The listing builds one solid part. Answer for the finished solid, in the listing's coordinates (mm). Face numbers are marked on the shaded views. Round coordinates to 2 decimals unless told otherwise and drop trailing zeros. Loops run counter-clockwise (first coordinate to the right, second up) from the corner with the lowest first, then second, coordinate; pieces in that order, holes last. Notation, with made-up numbers: (-10.75, 46.25) -> (11.25, 46.25) arc R12 ccw to (11.25, 66.25) -> close; hole circle Ø9 at (14, 89). An arc over 180 degrees is marked (long way). Write each question's results on one line, items separated by ' | '. Start each with the question number.
(1) A flat-ended cylindrical pin translates along its axis: pin 1 (0.6 mm diameter, centred on x = 2, y = -2.5, fed in from -Z). Find the tip coordinate at first contact, or state that the pin passes through.
(2) The part is cut by section C-C (y = 0). Determine the outline of the cut face in (x, z).
(3) The part is cut by section D-D (z = 10). Determine the outline of the cut face in (x, y), plus the area to 3 significant figures.
(4) The part is cut by section A-A (x = -7). Determine the outline of the cut face in (y, z), plus the area to 3 significant figures.
(5) Straight lines are drawn through the part: probe 1 along X at (y, z) = (-2.5, 10); probe 2 along X at (y, z) = (-1.5, -1.5); probe 3 along Z at (x, y) = (7.7, 0). For each, find the intervals that lie inside material, in ascending order.
(6) Determine the mould class of the marked faces 1, 2 and 3 for opening direction Y: released by +Y, released by -Y, zero draft, split by the parting line, or undercut.
(7) The part is cut by section B-B (z = 3.5). Determine the outline of the cut face in (x, y), plus the area to 3 significant figures.
```python
from build123d import *

# Parameters (mm, degrees)
SKETCH_1_R          = 2
EXTRUDE_1_DEPTH     = 12.5
SKETCH_2_R          = 1.7
CUT_EXTRUDE_1_DEPTH = 21.863604674
CUT_EXTRUDE_2_DEPTH = 6.5


with BuildPart() as part:
    # 草图1 → 凸台-拉伸1 (new, symmetric)
    with BuildSketch(Plane(origin=(0, 0, 0), x_dir=(0, 0, -1), z_dir=(1, 0, 0))):
        with BuildLine():
            Line((0, -3), (-16, -3))
            Line((-16, -3), (-16, -1.8))
            Line((-16, -1.8), (-2.4, -1.8))
            ThreePointArc((-2.4, -1.8), (1.341640786, 2.683281573), (0, -3))
        make_face()
        Circle(SKETCH_1_R, mode=Mode.SUBTRACT)
    extrude(amount=EXTRUDE_1_DEPTH, both=True)

    # 草图2 → 切除-拉伸1 (cut, through all)
    with BuildSketch(Plane(origin=(0, -1.8, 0), x_dir=(1, 0, 0), z_dir=(0, 1, 0))):
        with Locations(Location((-7, -10, 0), (0, 0, 270))):
            Circle(SKETCH_2_R)
        with Locations(Location((7, -10, 0), (0, 0, 270))):
            Circle(SKETCH_2_R)
    extrude(amount=-CUT_EXTRUDE_1_DEPTH, mode=Mode.SUBTRACT)

    # 草图3 → 切除-拉伸2 (cut, symmetric)
    with BuildSketch(Plane(origin=(0, 0, 0), x_dir=(0, 0, -1), z_dir=(1, 0, 0))):
        with BuildLine():
            Line((-4, -3), (0, -3))
            ThreePointArc((0, -3), (1.341640786, 2.683281573), (-2.4, -1.8))
            Line((-2.4, -1.8), (-4, -1.8))
            Line((-4, -1.8), (-4, -3))
        make_face()
    extrude(amount=CUT_EXTRUDE_2_DEPTH, both=True, mode=Mode.SUBTRACT)


solid = part.part
```
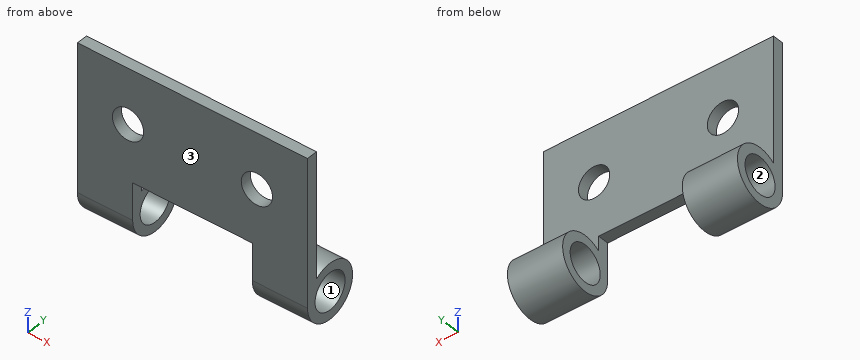
Checked values:
1) pin 1: stops at z = 4
2) outline: (-12.5, -3) -> (-6.5, -3) -> (-6.5, -2) -> (-12.5, -2) -> close; (-12.5, 2) -> (-6.5, 2) -> (-6.5, 3) -> (-12.5, 3) -> close; (6.5, -3) -> (12.5, -3) -> (12.5, -2) -> (6.5, -2) -> close; (6.5, 2) -> (12.5, 2) -> (12.5, 3) -> (6.5, 3) -> close
3) outline: (-12.5, -3) -> (-8.7, -3) -> (-8.7, -1.8) -> (-12.5, -1.8) -> close; (-5.3, -3) -> (5.3, -3) -> (5.3, -1.8) -> (-5.3, -1.8) -> close; (8.7, -3) -> (12.5, -3) -> (12.5, -1.8) -> (8.7, -1.8) -> close | area: 21.8 mm2
4) outline: (-3, 0) arc R3 ccw (long way) to (-1.8, 2.4) -> (-1.8, 8.3) -> (-3, 8.3) -> close; (-3, 11.7) -> (-1.8, 11.7) -> (-1.8, 16) -> (-3, 16) -> close; hole circle Ø4 at (0, 0) | area: 28.8 mm2
5) probe 1: x = -12.5 to -8.7, -5.3 to 5.3, 8.7 to 12.5 | probe 2: x = -12.5 to -6.5, 6.5 to 12.5 | probe 3: z = -3 to -2, 2 to 3
6) face 1: undercut | face 2: undercut | face 3: released by -Y
7) outline: (-12.5, -3) -> (-6.5, -3) -> (-6.5, -1.8) -> (-12.5, -1.8) -> close; (6.5, -3) -> (12.5, -3) -> (12.5, -1.8) -> (6.5, -1.8) -> close | area: 14.4 mm2
